Input: dimensioned drawing with shaded views. Units: mm. Origin: part minimum x, y, z. A direction names the side the tool comes from. Round coordinates to 2 decimals unless told otherwise and drop trailing zeros. Loops run counter-clockwise (first coordinate to the right, second up) from the corner with the lowest first, then second, coordinate; pieces in that order, holes last. Notation, with made-up numbers: M 3.5,46.5 L 28.5,46.5 A20 ccw 28.5,59.5 Z; hole C 29.5,63 d9. An arc over 180 degrees is marked long. Use one line per item in the form item = value. Start each with the question number.
Q1. Access query for the marked faces 1 and 2. Directions: +Z, -Z, +X, -X, +Y, -Y. A direction counts if a zero-diameter tool reaches every point of the face in a straight line with its end or side. Return the directions, or none.
Q2. Section query A-A, the plane x = 2.5. Output: boundary loops of the cut face in (y, z) (1 decimal), and give its area (3 significant figures).
Q3. First-contact query: P1, Ø4, axis at x = 10, y = 8.5, coming from the -Z side; P2, Ø1, axis at y = 3.5, z = 13.5, coming from the -X side; P3, Ø5, axis at x = 14, z = 4.5, coming from the +Y side. Flat tips, straight axial feed; report the tip coordinate or a pass-through.
Q4. Section query B-B, the plane x = 19.75. Output: boundary loops of the cut face in (y, z).
Q5. Ray query, line 1 along X through (y, z) = (15, 10); line 2 along X through (y, z) = (2.25, 11.75); line 3 along Z through (x, y) = (1.25, 2.75) (1 decimal). Return the intervals inside material, ascending.
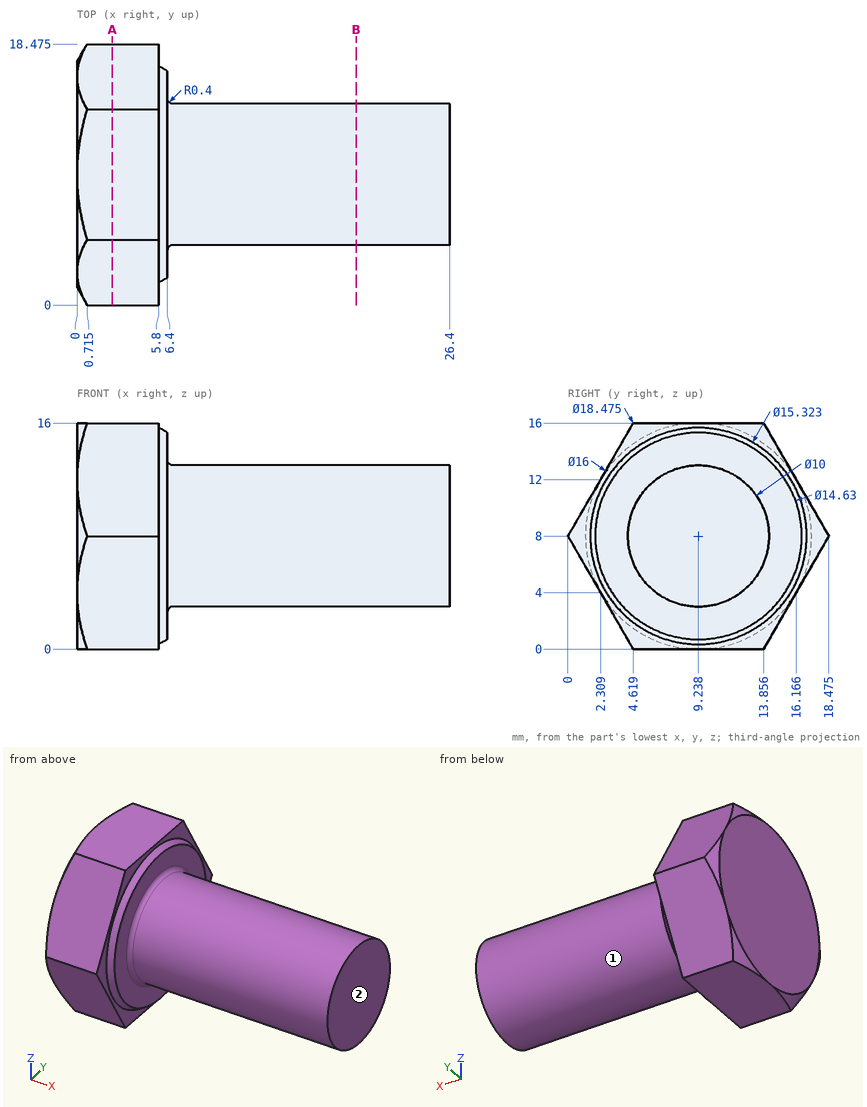
Results found:
q1.face_1 = +X
q1.face_2 = +Z, -Z, +X, +Y, -Y
q2.outline = M 0,8 L 4.6,0 L 13.9,0 L 18.5,8 L 13.9,16 L 4.6,16 Z
q2.area = 222 mm²
q3.P1 = 3
q3.P2 = 0
q3.P3 = 14.14
q4.outline = C 9.24,8 d10
q5.line_1 = 0 to 6.4
q5.line_2 = 0 to 5.8
q5.line_3 = 3.2 to 12.8
